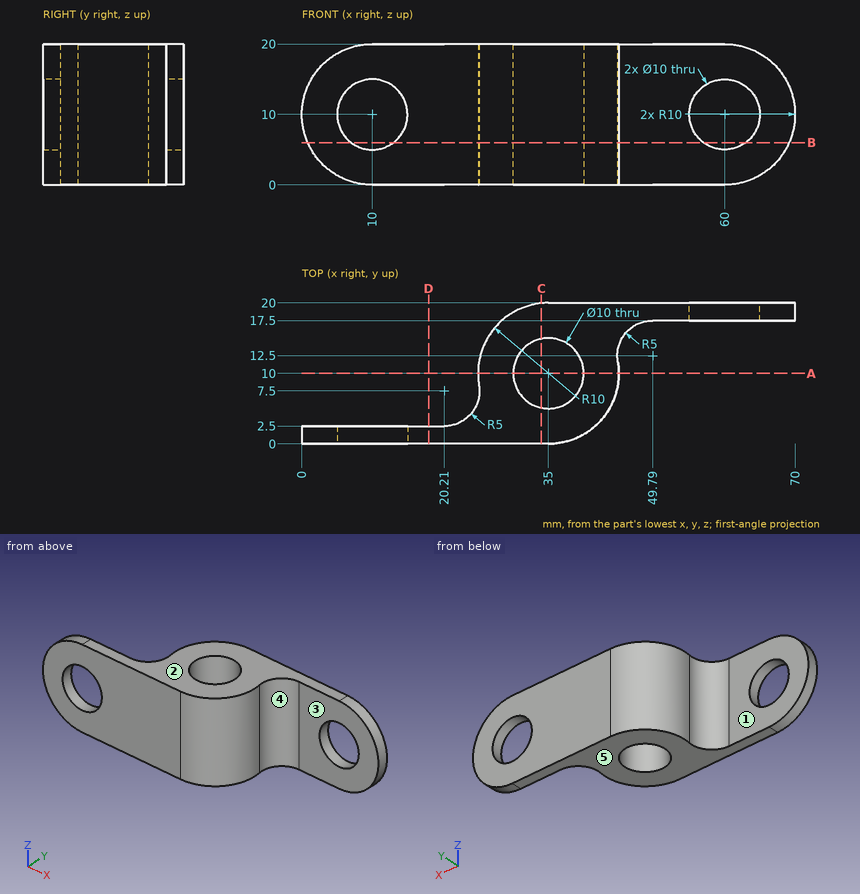
Here's the drawing with two shaded views (mm, measured from the low corner). I have some questions. A direction names the side the tool comes from. Give positions to 0.01 mm unless a question says otherwise; leave off trailing zeros. Write each loop counter-clockwise with the first axis right and the second up, starting at its lowest first coordinate (ties: lowest second). Pieces come first, ordered by that corner, then holes. Notation, with made-up numbers: (3.5, -22) - (59.5, -22) arc R18 cw to (59.5, 12) - close; hole circle Ø4 at (36.25, 16.5). An arc over 180 degrees is marked (long way). One line per item, written item: value. Start each with the question number.
Item 1: If we mould it in two halves opening along Y, with no side actions, what happens to the marked faces 3, 4 and 5? For each: +Y half, -Y half, draft (parallel to the pull), parting line (faces both ways), or undercut.
Item 2: Please list where these lines run through material, in increasing order: line 1 (Y direction, x = 64.5, z = 15.5); line 2 (X direction, y = 11.5, z = 1.5); line 3 (X direction, y = 6, z = 9.25) (1 decimal). Write a range as from..to.
Item 3: I'm going to push flat-ended pins straight in: pin 1 (6 mm diameter, centred on y = 11, z = 3, fed in from -X); pin 2 (5 mm diameter, centred on y = 16.5, z = 2.5, fed in from -X) (1 decimal); pin 3 (6 mm diameter, centred on x = 35, y = 10, fed in from -Z); pin 4 (12 mm diameter, centred on y = 17, z = 8, fed in from -X). Where does each tip first touch, or does it pass through?
Item 4: Imagine slicing it at A-A, the plane y = 10. List the corners of the cut face in (x, z) for me, and give its area (3 significant figures).
Item 5: Which directions (+Z, -Z, +X, -X, +Y, -Y) give clear straight access to the entire face, cutting with the end or side of a thin tool? Please do the marked faces 1 and 2.
Item 6: Imagine slicing it at C-C, the plane x = 34. List the corners of the cut face in (y, z) for me.
Item 7: Imagine slicing it at B-B, the plane z = 6. List the corners of the cut face in (x, y) for me (1 decimal).
Item 8: Imagine slicing it at D-D, the plane x = 18. List the corners of the cut face in (y, z) for me.
Geometry says:
1. face 3: -Y half
1. face 4: undercut
1. face 5: draft
2. line 1: 17.5..20
2. line 2: 25.11..30.23, 39.77..44.89
2. line 3: 25..32, 38..44.2
3. pin 1: x = 25
3. pin 2: x = 25.8
3. pin 3: through
3. pin 4: x = 25.05
4. outline: (25, 0) - (30, 0) - (30, 20) - (25, 20) - close; (40, 0) - (45, 0) - (45, 20) - (40, 20) - close
4. area: 200 mm^2
5. face 1: +Z, -Z, -X, +Y
5. face 2: +Z, +X, -X, +Y, -Y
6. outline: (0, 0) - (5.1, 0) - (5.1, 20) - (0, 20) - close; (14.9, 0) - (19.95, 0) - (19.95, 20) - (14.9, 20) - close
7. outline: (0.8, 0) - (7, 0) - (7, 2.5) - (0.8, 2.5) - close; (13, 0) - (35, 0) arc R10 ccw to (44.9, 11.7) arc R5 cw to (49.8, 17.5) - (57, 17.5) - (57, 20) - (35, 20) arc R10 ccw to (25.1, 8.3) arc R5 cw to (20.2, 2.5) - (13, 2.5) - close; (63, 17.5) - (69.2, 17.5) - (69.2, 20) - (63, 20) - close; hole circle Ø10 at (35, 10)
8. outline: (0, 0) - (2.5, 0) - (2.5, 20) - (0, 20) - close
